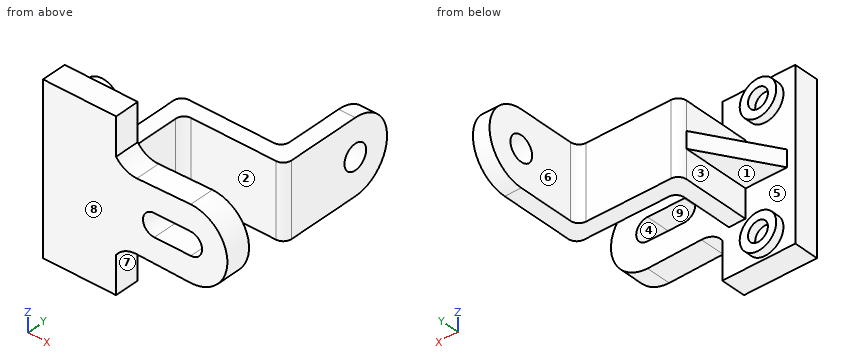
from build123d import *

# Parameters (mm, degrees)
BRACKET_PROFILE_SKETCH_W = 44
BRACKET_PROFILE_SKETCH_H = 15
BRACKET_BASE_BODY_DEPTH  = 50
UPRIGHT_WEB_DEPTH        = 22
LUG_BOSS_DEPTH           = 10
LUG_HOLE_CUT_DEPTH       = 44
WASHER_BOSS_SKETCH_R     = 11
WASHER_BOSS_SKETCH_R_2   = 6
WASHER_BOSS_22_DEPTH     = 5
WEB_PAD_DEPTH            = 5
SLOTTED_TAB_DEPTH        = 15


with BuildPart() as part:
    # Bracket Profile Sketch → Bracket Base Body (new, symmetric)
    with BuildSketch(Plane.XY):
        Rectangle(BRACKET_PROFILE_SKETCH_W, BRACKET_PROFILE_SKETCH_H)
    extrude(amount=BRACKET_BASE_BODY_DEPTH, both=True)

    # Sketch1_3 → Upright Web (add, symmetric)
    with BuildSketch(Plane.XY):
        with BuildLine():
            Line((8, 7.5), (18, 7.5))
            Line((18, 7.5), (18, 38.383152955))
            ThreePointArc((18, 38.383152955), (19.464466094, 41.91868686), (23, 43.383152955))
            Line((23, 43.383152955), (74.071731591, 43.383152955))
            ThreePointArc((74.071731591, 43.383152955), (77.607265497, 44.847619049), (79.071731591, 48.383152955))
            Line((79.071731591, 48.383152955), (79.071731591, 92.5))
            Line((79.071731591, 92.5), (69.071731591, 92.5))
            Line((69.071731591, 92.5), (69.071731591, 58.383152955))
            ThreePointArc((69.071731591, 58.383152955), (67.607265497, 54.847619049), (64.071731591, 53.383152955))
            Line((64.071731591, 53.383152955), (13, 53.383152955))
            ThreePointArc((13, 53.383152955), (9.464466094, 51.91868686), (8, 48.383152955))
            Line((8, 48.383152955), (8, 7.5))
        make_face()
    extrude(amount=UPRIGHT_WEB_DEPTH, both=True)

    # Lug Profile Sketch → Lug Boss (add)
    with BuildSketch(Plane.ZY.offset(-69.071731591)):
        with BuildLine():
            Line((7.5, 92.5), (22, 92.5))
            ThreePointArc((22, 92.5), (0, 114.5), (-22, 92.5))
            Line((-22, 92.5), (-7.5, 92.5))
            ThreePointArc((-7.5, 92.5), (0, 100), (7.5, 92.5))
        make_face()
    extrude(amount=-LUG_BOSS_DEPTH)

    # Sketch2_3 → Lug Hole Cut (cut)
    with BuildSketch(Plane.ZY.offset(-69.071731591)):
        with BuildLine():
            ThreePointArc((-7.5, 92.5), (0, 85), (7.5, 92.5))
            Line((7.5, 92.5), (-7.5, 92.5))
        make_face()
        with BuildLine():
            Line((-7.5, 92.5), (7.5, 92.5))
            ThreePointArc((7.5, 92.5), (0, 100), (-7.5, 92.5))
        make_face()
    extrude(amount=-LUG_HOLE_CUT_DEPTH, mode=Mode.SUBTRACT)

    # Washer Boss Sketch → Washer Boss _22 (add)
    # profile 1 of 2: a face of its own
    with BuildSketch(Plane(origin=(0, 7.5, 0), x_dir=(1, 0, 0), z_dir=(0, 1, 0))):
        with Locations((-3.843200035, 37.271330251)):
            Circle(WASHER_BOSS_SKETCH_R)
        with Locations(Location((-3.843200035, 37.271330251, 0), (0, 0, 180))):
            Circle(WASHER_BOSS_SKETCH_R_2, mode=Mode.SUBTRACT)
    # profile 2 of 2: a face of its own
    with BuildSketch(Plane(origin=(0, 7.5, 0), x_dir=(1, 0, 0), z_dir=(0, 1, 0))):
        with Locations((-3.843200035, -37.271330251)):
            Circle(WASHER_BOSS_SKETCH_R)
        with Locations((-3.843200035, -37.271330251)):
            Circle(WASHER_BOSS_SKETCH_R_2, mode=Mode.SUBTRACT)
    extrude(amount=WASHER_BOSS_22_DEPTH)

    # Web Pad Sketch → Web Pad (add, symmetric)
    with BuildSketch(Plane.XY):
        Polygon((8, 48.383152955), (-17, 7.5), (8, 7.5), align=None)
    extrude(amount=WEB_PAD_DEPTH, both=True)

    # Slotted Tab Sketch → Slotted Tab (add)
    with BuildSketch(Plane.XZ.offset(7.5)):
        with BuildLine():
            Line((66.991803694, 21.999998473), (34.541419601, 21.210572784))
            ThreePointArc((34.541419601, 21.210572784), (27.498169269, 22.774892965), (22, 27.446574412))
            Line((22, 27.446574412), (22, -27.446574412))
            ThreePointArc((22, -27.446574412), (27.498169269, -22.774892965), (34.541419601, -21.210572784))
            Line((34.541419601, -21.210572784), (66.991803694, -21.999998473))
            ThreePointArc((66.991803694, -21.999998473), (89, 0), (66.991803694, 21.999998473))
        make_face()
        with BuildLine():
            ThreePointArc((67, 6.793312715), (73.793312715, 0), (67, -6.793312715))
            Line((67, -6.793312715), (45, -6.793312715))
            ThreePointArc((45, -6.793312715), (38.206687285, 0), (45, 6.793312715))
            Line((45, 6.793312715), (67, 6.793312715))
        make_face(mode=Mode.SUBTRACT)
    extrude(amount=-SLOTTED_TAB_DEPTH)


solid = part.part
The model under review builds one solid part; all positions refer to its coordinate system, in mm. Face numbers are marked on the shaded views. A direction names the side the tool comes from. Give positions to 0.01 mm unless a question says otherwise; leave off trailing zeros. Order: outer loops, then holes, each group sorted by start corner. A loop starts at its lowest first (then second) coordinate and runs counter-clockwise, first axis right, second up. Notation, with made-up numbers: M 33,27 L 87,27 A18 cw 87,47 Z; hole C 19,89.5 d6. An arc over 180 degrees is marked long. Answer in a Markdown table with one row per item. Add a question column.
1. Add section A-A on z = 0. State the section outline as (x, y) points, plus the area to 3 significant figures.
2. To check wall thickness, follow line 1 along Y through (x, z) = (71, 0); line 2 along Y through (x, z) = (47, -11); line 3 along Y through (x, z) = (-4, -39.5). State the ranges of each line that lie inside material, in increasing order.
3. Add section C-C on y = 22. State the section outline as (x, z) points, plus the area to 3 significant figures.
4. Machinability: for the marked faces 1, 2, 3, 4 and 5, which of the approach directions +Z, -Z, +X, -X, +Y, -Y give a long, thin tool a straight path to every point of the face, cutting with its end or side? Answer none if there is none.
5. Mouldability with a two-part tool opening along X and no side actions: class the marked faces 6, 7, 8 and 9 as released by +X, released by -X, zero draft, split by the parting line, or undercut.
6. Add section B-B on x = 41. State the section outline as (y, z) points, plus the area to 3 significant figures.
7. Add section D-D on x = 5. State the section outline as (y, z) points, plus the area to 3 significant figures.
8. For pin 1 Ø8.5 at (y, z) = (22, 12) entering from -X; pin 2 Ø12 at (y, z) = (77, 25) entering from -X; pin 3 Ø16.5 at (x, y) = (51, -3) entering from +Z; pin 4 Ø21.5 at (x, y) = (33.5, 65.5) entering from +Z (3 decimals), all flat-tipped, find the tip position at first contact; note any pin that passes through.
The answers:
| question | item | result |
|---|---|---|
| 1 | outline | M -22,-7.5 L 38.21,-7.5 L 38.21,7.5 L 18,7.5 L 18,38.38 A5 cw 23,43.38 L 74.07,43.38 A5 ccw 79.07,48.38 L 79.07,85 L 69.07,85 L 69.07,58.38 A5 cw 64.07,53.38 L 13,53.38 A5 ccw 8,48.38 L -17,7.5 L -22,7.5 Z; M 69.07,100 L 79.07,100 L 79.07,114.5 L 69.07,114.5 Z; M 73.79,-7.5 L 89,-7.5 L 89,7.5 L 73.79,7.5 Z |
| 1 | area | 3,170 mm2 |
| 2 | line 1 | 43.38 to 85, 100 to 114.5 |
| 2 | line 2 | -7.5 to 7.5, 43.38 to 53.38 |
| 2 | line 3 | -7.5 to 7.5 |
| 3 | outline | M -8.13,-5 L 8,-5 L 8,-22 L 18,-22 L 18,22 L 8,22 L 8,5 L -8.13,5 Z |
| 3 | area | 601 mm2 |
| 4 | face 1 | -X, +Y |
| 4 | face 2 | +Z, -Z, +X |
| 4 | face 3 | -Z, -X, +Y |
| 4 | face 4 | -Y |
| 4 | face 5 | none |
| 5 | face 6 | released by -X |
| 5 | face 7 | released by +X |
| 5 | face 8 | zero draft |
| 5 | face 9 | undercut |
| 6 | outline | M -7.5,-21.37 L 7.5,-21.37 L 7.5,-5.49 L -7.5,-5.49 Z; M -7.5,5.49 L 7.5,5.49 L 7.5,21.37 L -7.5,21.37 Z; M 43.38,-22 L 53.38,-22 L 53.38,22 L 43.38,22 Z |
| 6 | area | 916 mm2 |
| 7 | outline | M -7.5,-50 L 7.5,-50 L 7.5,-43.81 L 12.5,-43.81 L 12.5,-30.73 L 7.5,-30.73 L 7.5,-5 L 43.48,-5 L 43.48,5 L 7.5,5 L 7.5,30.73 L 12.5,30.73 L 12.5,43.81 L 7.5,43.81 L 7.5,50 L -7.5,50 Z |
| 7 | area | 1,990 mm2 |
| 8 | pin 1 | x = 8 |
| 8 | pin 2 | x = 69.07 |
| 8 | pin 3 | z = 21.81 |
| 8 | pin 4 | through |
